Geometry: final body of the model. Coordinates: model frame, mm. A direction names the side the tool comes from. Round coordinates to 2 decimals unless told otherwise and drop trailing zeros. Order: outer loops, then holes, each group sorted by start corner. A loop starts at its lowest first (then second) coordinate and runs counter-clockwise, first axis right, second up. Notation, with made-up numbers: M 75.5,44.5 L 121.5,44.5 A19 cw 121.5,49.5 Z; hole C -18.5,11.25 d2. An arc over 180 degrees is marked long. Put each result on its own line as item: value. Start each with the question number.
1) Section C-C, the plane y = -43. Return loops of the section in (x, z), then the cut area to 3 significant figures.
2) Section B-B, the plane x = 0. Return loops of the section in (y, z).
3) First-contact query: P1, Ø3, axis at x = 23, y = -30.5, coming from the +Z side; P2, Ø3, axis at x = 18, z = 23.5, coming from the -Y side; P3, Ø10, axis at x = -19, y = -69.5, coming from the -Z side. Flat tips, straight axial feed; report the tip coordinate or a pass-through.
4) Draft query along Z for faces 6 (the flat face through (0, -20, -18.65)), 7 (the flat face through (-15, -31, -26)), 8 (the cylindrical face through (16.65, -30.68, -19.32)). Return one class per face: pulls with the +Z half, pulls with the -Z half, needs draft (parallel to the pull), parting line crosses it, or undercut.
5) Section A-A, the plane z = 0. Return loops of the section in (x, y), then the cut area to 3 significant figures.
6) Access query for faces 1 (the flat face through (21, -32.1, -23)), 2 (the flat face through (-24.5, -28.8, -20.8)), 3 (the flat face through (-20, -32.1, 23)), 4 (the flat face through (23, -31, 17.75)), 5 (the flat face through (0, -21.5, -24)). Directions: +Z, -Z, +X, -X, +Y, -Y. A direction counts if a zero-diameter tool reaches every point of the face in a straight line with its end or side. Return the directions, or none.
7) Section D-D, the plane z = -16. Return loops of the section in (x, y).
8) Material intervals for probe 1 along Y at (x, z) = (-6.5, -24.5); probe 2 along Y at (x, z) = (-14, -17.5); probe 3 along Z at (x, y) = (-10.5, -72.5), sorted ascending. Write a range as [from, to].
from build123d import *

# Parameters (mm, degrees)
EXTRUDE_1_DEPTH             = 26.5
EXTRUDE_1_DEPTH_BACK        = 26.5
SKETCH_2_W                  = 57
SKETCH_2_H                  = 61
CUT_EXTRUDE_1_DEPTH         = 32.5
EXTRUDE_2_DEPTH             = 2
SKETCH_5_W                  = 57
SKETCH_5_H                  = 61
CUT_EXTRUDE_2_DEPTH         = 3.7
PATTERN_LINEAR_1_COUNT      = 2
PATTERN_LINEAR_1_PITCH      = 46.5
PATTERN_LINEAR_1_COUNT_DIR2 = 2
PATTERN_LINEAR_1_PITCH_DIR2 = 41


with BuildPart() as part:
    # 草图1 → 凸台-拉伸1 (new, two sides: drawn at the far end of the back side and taken through both)
    with BuildSketch(Plane(origin=(0, 0, 0), x_dir=(0, 0, -1), z_dir=(1, 0, 0)).offset(-EXTRUDE_1_DEPTH_BACK)):
        Polygon((-28.5, -32.5), (28.5, -32.5), (28.5, -21.5), (18.65, -21.5), (18.65, -19.3), (-18.65, -19.3), (-18.65, -21.5), (-28.5, -21.5), align=None)
    extrude(amount=EXTRUDE_1_DEPTH + EXTRUDE_1_DEPTH_BACK)

    # 草图2 → 切除-拉伸1 (cut)
    with BuildSketch(Plane(origin=(0, 0, 0), x_dir=(1, 0, 0), z_dir=(0, 1, 0))):
        Rectangle(SKETCH_2_W, SKETCH_2_H)
        with BuildLine():
            Line((-26.5, -15), (-25.638357139, -24.848622971))
            ThreePointArc((-25.638357139, -24.848622971), (-24.355939177, -27.449109347), (-21.653578346, -28.5))
            Line((-21.653578346, -28.5), (21.653578346, -28.5))
            ThreePointArc((21.653578346, -28.5), (24.355939177, -27.449109347), (25.638357139, -24.848622971))
            Line((25.638357139, -24.848622971), (26.5, -15))
            Line((26.5, -15), (26.5, 15))
            Line((26.5, 15), (25.638357139, 24.848622971))
            ThreePointArc((25.638357139, 24.848622971), (24.355939177, 27.449109347), (21.653578346, 28.5))
            Line((21.653578346, 28.5), (-21.653578346, 28.5))
            ThreePointArc((-21.653578346, 28.5), (-24.355939177, 27.449109347), (-25.638357139, 24.848622971))
            Line((-25.638357139, 24.848622971), (-26.5, 15))
            Line((-26.5, 15), (-26.5, -15))
        make_face(mode=Mode.SUBTRACT)
    extrude(amount=-CUT_EXTRUDE_1_DEPTH, mode=Mode.SUBTRACT)

    # 草图3 → 旋转1 (revolve)
    with BuildSketch(Plane.XY, mode=Mode.PRIVATE) as revolve_1_sk:
        Polygon((0, -32.5), (22.5, -32.5), (22.5, -50.5), (21.5, -50.5), (21.5, -83.5), (0, -83.5), align=None)
    revolve(revolve_1_sk.sketch.rotate(Axis((0, -83.5, 0), (0, 1, 0)), 270), axis=Axis((0, -83.5, 0), (0, 1, 0)))

    # 草图4 → 凸台-拉伸2 (add)
    with BuildSketch(Plane(origin=(0, -32.5, 0), x_dir=(1, 0, 0), z_dir=(0, 1, 0))):
        with BuildLine():
            Line((-22.5, -2.9), (-19.5, -2.9))
            Line((-19.5, -2.9), (-19.5, 2.9))
            Line((-19.5, 2.9), (-22.5, 2.9))
            ThreePointArc((-22.5, 2.9), (-25.4, 0), (-22.5, -2.9))
        make_face()
    extrude(amount=-EXTRUDE_2_DEPTH)

    # 草图5 → 切除-拉伸2 (cut)
    with BuildSketch(Plane(origin=(0, -32.5, 0), x_dir=(1, 0, 0), z_dir=(0, 1, 0))):
        Rectangle(SKETCH_5_W, SKETCH_5_H)
        with BuildLine():
            Line((-26.5, -17.75), (-20.5, -17.75))
            ThreePointArc((-20.5, -17.75), (-16.610912703, -19.360912703), (-15, -23.25))
            Line((-15, -23.25), (-15, -28.5))
            Line((-15, -28.5), (15, -28.5))
            Line((15, -28.5), (15, -23.25))
            ThreePointArc((15, -23.25), (16.610912703, -19.360912703), (20.5, -17.75))
            Line((20.5, -17.75), (26.5, -17.75))
            Line((26.5, -17.75), (26.5, 17.75))
            Line((26.5, 17.75), (20.5, 17.75))
            ThreePointArc((20.5, 17.75), (16.610912703, 19.360912703), (15, 23.25))
            Line((15, 23.25), (15, 28.5))
            Line((15, 28.5), (-15, 28.5))
            Line((-15, 28.5), (-15, 23.25))
            ThreePointArc((-15, 23.25), (-16.610912703, 19.360912703), (-20.5, 17.75))
            Line((-20.5, 17.75), (-26.5, 17.75))
            Line((-26.5, 17.75), (-26.5, -17.75))
        make_face(mode=Mode.SUBTRACT)
    extrude(amount=CUT_EXTRUDE_2_DEPTH, mode=Mode.SUBTRACT)

    # 草图6 → 旋转2 (revolve)
    with BuildSketch(Plane.XY.offset(23.25), mode=Mode.PRIVATE) as revolve_2_sk:
        with BuildLine():
            Line((20.5, -28.8), (25, -28.8))
            Line((25, -28.8), (25, -30.5))
            ThreePointArc((25, -30.5), (24.53137085, -31.63137085), (23.4, -32.1))
            Line((23.4, -32.1), (20.5, -32.1))
            Line((20.5, -32.1), (20.5, -28.8))
        make_face()
    revolve_2 = revolve(revolve_2_sk.sketch.rotate(Axis((20.5, -32.1, 23.25), (0, 1, 0)), 270), axis=Axis((20.5, -32.1, 23.25), (0, 1, 0)))

    # 阵列(线性)1: Revolve 2 2 × 2
    with Locations(*[(-j * PATTERN_LINEAR_1_PITCH_DIR2, 0, -i * PATTERN_LINEAR_1_PITCH) for i in range(PATTERN_LINEAR_1_COUNT) for j in range(PATTERN_LINEAR_1_COUNT_DIR2) if (i, j) != (0, 0)]):
        add(revolve_2)


solid = part.part
Result sheet:
1. outline: C 0,0 d45
1. area: 1,590 mm2
2. outline: M -83.5,-21.5 L -50.5,-21.5 L -50.5,-22.5 L -32.5,-22.5 L -32.5,-28.5 L -21.5,-28.5 L -21.5,-18.65 L -19.3,-18.65 L -19.3,18.65 L -21.5,18.65 L -21.5,28.5 L -32.5,28.5 L -32.5,22.5 L -50.5,22.5 L -50.5,21.5 L -83.5,21.5 Z
3. P1: stops at z = 27.64
3. P2: stops at y = -32.1
3. P3: stops at z = -16.32
4. face 6: pulls with the -Z half
4. face 7: needs draft
4. face 8: undercut
5. outline: M -26.5,-32.5 L -25.4,-32.5 L -25.4,-34.5 L -22.5,-34.5 L -22.5,-50.5 L -21.5,-50.5 L -21.5,-83.5 L 21.5,-83.5 L 21.5,-50.5 L 22.5,-50.5 L 22.5,-32.5 L 26.5,-32.5 L 26.5,-19.3 L -26.5,-19.3 Z
5. area: 2,930 mm2
6. face 1: -Z, +X, -Y
6. face 2: -Y
6. face 3: +Z, -X, -Y
6. face 4: +X, -Y
6. face 5: -Z, +X, -X, +Y
7. outline: M -26.41,-32.5 L -15.82,-32.5 L -15.82,-50.5 L -14.36,-50.5 L -14.36,-83.5 L 14.36,-83.5 L 14.36,-50.5 L 15.82,-50.5 L 15.82,-32.5 L 26.41,-32.5 L 26.41,-19.3 L -26.41,-19.3 Z
8. probe 1: y = [-32.5, -21.5]
8. probe 2: y = [-50.5, -19.3]
8. probe 3: z = [-18.76, 18.76]
